Work out the finished part from the listing and answer in its coordinate system (mm). A direction names the side the tool comes from. Coordinates: 2 decimals unless noted, no trailing zeros. Write each loop counter-clockwise with the first axis right and the second up, starting at its lowest first coordinate (ties: lowest second). Pieces come first, ordered by that corner, then holes. Notation, with made-up numbers: M 16.5,-3 L 46.5,-3 A35 ccw 46.5,34 Z; hole C 25,39.5 d9. An arc over 180 degrees is marked long. Answer as CSV lines item,"result". Start each with the question number.
(1) Flat-ended cylindrical pins translate along their axes: P1, Ø4, axis at y = -37.5, z = 14.5, coming from the +X side; P2, Ø12, axis at x = 29.5, z = 19.5, coming from the +Y side; P3, Ø8, axis at x = 72.5, z = 13.5, coming from the -Y side; P4, Ø5, axis at y = 2.5, z = 13, coming from the +X side. Find the tip coordinate at first contact, or state that the pin passes through.
(2) For faces 1 (the flat face through (100.29, 46.84, 17.55)), 2 (the cylindrical face through (257.987, 1.133, 17.551)), determine the directions among +Z, -Z, +X, -X, +Y, -Y from which every point of the face is accessible in a straight line to the end or side of a thin tool.
(3) A cutting plane is placed at B-B on z = 28. Give the vertices of the cut face in (x, y).
(4) A cutting plane is placed at C-C on x = 216. Give the vertices of the cut face in (y, z).
(5) Find the intervals of material crossed by L1, parallel to X at y = 2, z = 21; L2, parallel to Y at x = 115, z = 15; L3, parallel to Y at x = 224, z = 32, in increasing order. Write a range as [from, to].
(6) A cutting plane is placed at A-A on y = 0. Give the vertices of the cut face in (x, z).
(7) The mould has two halves that part along X. Classify faces 3 (the cylindrical face through (-39.99, -0.85, 17.55)), 4 (the flat face through (110, -46, 35.6)), 5 (the flat face through (103.19, -46.98, 17.55)): released by +X, released by -X, zero draft, split by the parting line, or undercut.
from build123d import *

# Parameters (mm, degrees)
BOSS_EXTRUDE1_DEPTH = 35.6


with BuildPart() as part:
    # Sketch1 → Boss-Extrude1 (new body)
    with BuildSketch(Plane.XY):
        with BuildLine():
            Line((-2.017486069, 41.915184916), (205.5017447, 51.903621277))
            ThreePointArc((205.5017447, 51.903621277), (259.963710234, 0), (205.5017447, -51.903621277))
            Line((205.5017447, -51.903621277), (-2.017486069, -41.915184916))
            ThreePointArc((-2.017486069, -41.915184916), (-41.963710234, 0), (-2.017486069, 41.915184916))
        make_face()
        with BuildLine():
            Line((-1.923076923, 39.953745446), (205.596153846, 49.942181807))
            ThreePointArc((205.596153846, 49.942181807), (258, 0), (205.596153846, -49.942181807))
            Line((205.596153846, -49.942181807), (-1.923076923, -39.953745446))
            ThreePointArc((-1.923076923, -39.953745446), (-40, 0), (-1.923076923, 39.953745446))
        make_face(mode=Mode.SUBTRACT)
    extrude(amount=BOSS_EXTRUDE1_DEPTH)


solid = part.part
Here are the results:
1,P1,"stops at x = 245.95"
1,P2,"stops at y = 43.72"
1,P3,"stops at y = -45.69"
1,P4,"stops at x = 259.96"
2,face 1,"+Z, -Z, -X, +Y"
2,face 2,"+Z, -Z"
3,outline,"M -2.02,-41.92 L 205.5,-51.9 A51.96 ccw long 205.5,51.9 L -2.02,41.92 A41.96 ccw Z; hole M -1.92,-39.95 L 205.6,-49.94 A50 ccw long 205.6,49.94 L -1.92,39.95 A40 ccw Z"
4,outline,"M -51.34,0 L -49.36,0 L -49.36,35.6 L -51.34,35.6 Z; M 49.36,0 L 51.34,0 L 51.34,35.6 L 49.36,35.6 Z"
5,L1,"x = [-41.92, -39.95], [257.96, 259.93]"
5,L2,"y = [-47.55, -45.58], [45.58, 47.55]"
5,L3,"y = [-49.44, -47.37], [47.37, 49.44]"
6,outline,"M -41.96,0 L -40,0 L -40,35.6 L -41.96,35.6 Z; M 258,0 L 259.96,0 L 259.96,35.6 L 258,35.6 Z"
7,face 3,"undercut"
7,face 4,"zero draft"
7,face 5,"released by -X"
